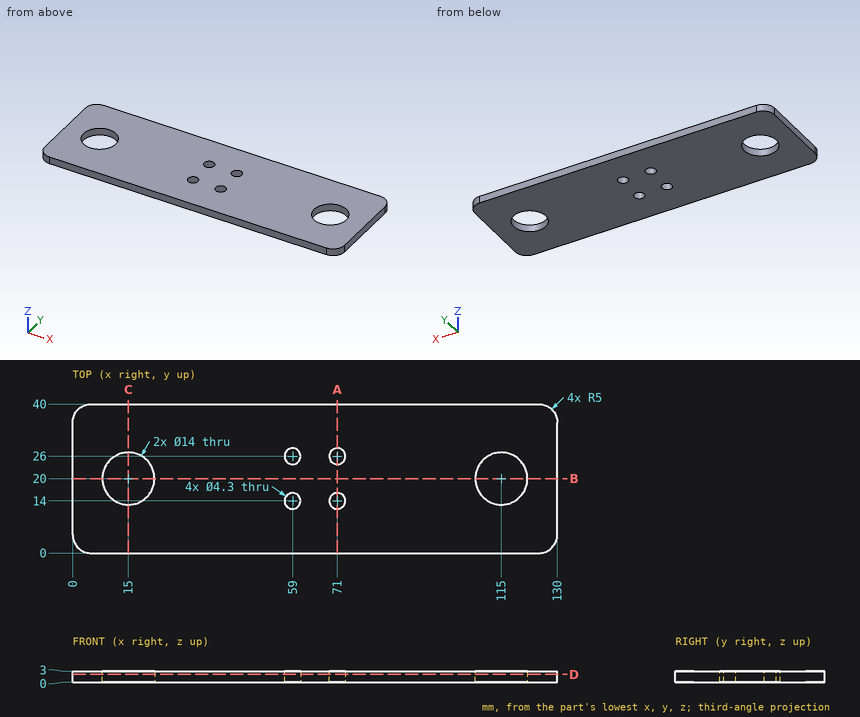
The figure shows three views and two pictorial views of one solid part (mm, origin at its lowest corner). Answer the questions. Give positions to 0.01 mm unless a question says otherwise; leave off trailing zeros. Order: outer loops, then holes, each group sorted by start corner. A loop starts at its lowest first (then second) coordinate and runs counter-clockwise, first axis right, second up. Notation, with made-up numbers: (-11, 6.25) - (31, 6.25) arc R33 cw to (31, 38.25) - close; hole circle Ø11 at (-25, 29). An arc over 180 degrees is marked (long way). Answer as CSV lines item,"result".
Q1. A cutting plane is placed at B-B, the plane y = 20. Determine the outline of the cut face in (x, z).
Answer key:
outline,"(0, 0) - (8, 0) - (8, 3) - (0, 3) - close; (22, 0) - (108, 0) - (108, 3) - (22, 3) - close; (122, 0) - (130, 0) - (130, 3) - (122, 3) - close"
Q2. A cutting plane is placed at D-D, the plane z = 2.15. Determine the outline of the cut face in (x, y).
Answer key:
outline,"(0, 5) arc R5 ccw to (5, 0) - (125, 0) arc R5 ccw to (130, 5) - (130, 35) arc R5 ccw to (125, 40) - (5, 40) arc R5 ccw to (0, 35) - close; hole circle Ø14 at (15, 20); hole circle Ø4.3 at (59, 14); hole circle Ø4.3 at (59, 26); hole circle Ø4.3 at (71, 14); hole circle Ø4.3 at (71, 26); hole circle Ø14 at (115, 20)"
Q3. A cutting plane is placed at C-C, the plane x = 15. Determine the outline of the cut face in (y, z), and give its area (3 significant figures).
Answer key:
outline,"(0, 0) - (13, 0) - (13, 3) - (0, 3) - close; (27, 0) - (40, 0) - (40, 3) - (27, 3) - close"
area,"78.0 mm^2"
Q4. Straight lines are drawn through the part: L1, parallel to Y at x = 59, z = 2.2; L2, parallel to X at y = 17, z = 2.85; L3, parallel to X at y = 24.5, z = 2.4. For each, find the intervals that lie inside material, in ascending order.
Answer key:
L1,"y = 0 to 11.85, 16.15 to 23.85, 28.15 to 40"
L2,"x = 0 to 8.68, 21.32 to 108.68, 121.32 to 130"
L3,"x = 0 to 9.64, 20.36 to 57.46, 60.54 to 69.46, 72.54 to 109.64, 120.36 to 130"
Q5. A cutting plane is placed at A-A, the plane x = 71. Determine the outline of the cut face in (y, z), and give its area (3 significant figures).
Answer key:
outline,"(0, 0) - (11.85, 0) - (11.85, 3) - (0, 3) - close; (16.15, 0) - (23.85, 0) - (23.85, 3) - (16.15, 3) - close; (28.15, 0) - (40, 0) - (40, 3) - (28.15, 3) - close"
area,"94.2 mm^2"
